from build123d import *

# Parameters (mm, degrees)
SKETCH1_R           = 28
BOSS_EXTRUDE1_DEPTH = 15
HOLE1_D             = 17
HOLE2_D             = 5.5
HOLE2_CBORE_D       = 10
HOLE2_CBORE_DEPTH   = 7
CHAMFER1_SIZE       = 1


with BuildPart() as part:
    # Sketch1 → Boss-Extrude1 (new body)
    with BuildSketch(Plane.XY):
        Circle(SKETCH1_R)
    extrude(amount=BOSS_EXTRUDE1_DEPTH)

    # Hole1 (through all)
    with Locations(Plane.XY.offset(15)):
        with Locations((0, 0)):
            Hole(HOLE1_D / 2)

    # Hole2 (through all)
    with Locations(Plane.XY.offset(15)):
        with Locations((-20, 0), (20, 0)):
            CounterBoreHole(HOLE2_D / 2, HOLE2_CBORE_D / 2, HOLE2_CBORE_DEPTH)

    # Chamfer1
    chamfer1_edges = [part.edges().sort_by_distance(p)[0] for p in [
        (-28, 0, 0),
        (-28, 0, 15),
        (8.5, 0, 15),
        (8.5, 0, 0),
    ]]
    chamfer(chamfer1_edges, length=CHAMFER1_SIZE)


solid = part.part
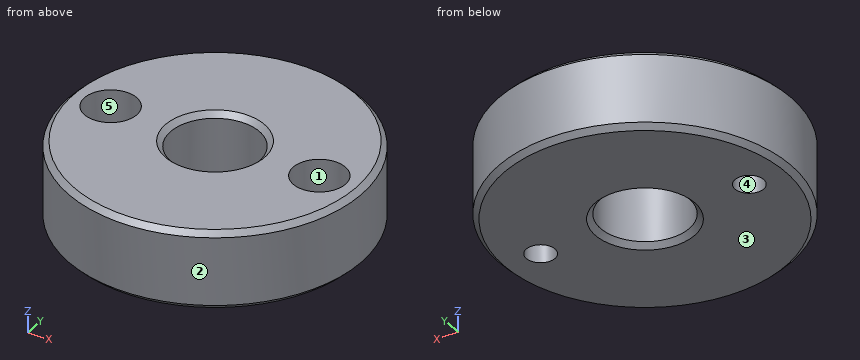
For this review, take the finished solid that the model builds, in its own axes (mm). Face numbers are marked on the shaded views. A direction names the side the tool comes from. Give positions to 0.01 mm unless a question says otherwise; leave off trailing zeros. Loops run counter-clockwise (first coordinate to the right, second up) from the corner with the lowest first, then second, coordinate; pieces in that order, holes last.
Item 1: For line 1 along Y through (x, z) = (0, 8.5); line 2 along X through (y, z) = (7.5, 9.5); line 3 along Y through (x, z) = (-20, 12), list the stretches that pass through material, from the lowest coordinate up.
Item 2: Draft analysis for pull direction X (two halves, no side actions). For the marked faces 1, 2 and 3, state which applies: +X half, -X half, draft (parallel to the pull), parting line (faces both ways), or undercut.
Item 3: Take a section at B-B, the plane x = 0. State the section outline as (y, z) points, and give its area (3 significant figures).
Item 4: Take a section at C-C, the plane z = 11. State the section outline as (x, y) points, and give its area (3 significant figures).
Item 5: Tool access review of the marked faces 4 and 5: name each direction out of +Z, -Z, +X, -X, +Y, -Y from which nothing blocks a thin tool from reaching the whole face with its end or side.
Item 6: Take a section at A-A, the plane y = 0. Give the number of separate pieces and of enclosed holes in the cut face, and give its area (3 significant figures).
Item 7: Insertion check: pin 1 (6.5 mm diameter, centred on x = -20, y = 0, fed in from +Z); pin 2 (3 mm diameter, centred on y = -12, z = 10.5, fed in from -X); pin 3 (2 mm diameter, centred on y = 2.5, z = 1.5, fed in from -X). Each pin has a flat end and moves straight along its axis. Give the tip position at first contact, or say it passes through.
Calculated:
1. line 1: y = -28 to -8.5, 8.5 to 28
1. line 2: x = -26.98 to -4, 4 to 26.98
1. line 3: y = -19.6 to -5, 5 to 19.6
2. face 1: undercut
2. face 2: parting line
2. face 3: draft
3. outline: (-28, 1) - (-27, 0) - (-9.5, 0) - (-8.5, 1) - (-8.5, 14) - (-9.5, 15) - (-27, 15) - (-28, 14) - close; (8.5, 1) - (9.5, 0) - (27, 0) - (28, 1) - (28, 14) - (27, 15) - (9.5, 15) - (8.5, 14) - close
3. area: 581 mm2
4. outline: circle Ø56 at (0, 0); hole circle Ø10 at (-20, 0); hole circle Ø17 at (0, 0); hole circle Ø10 at (20, 0)
4. area: 2,080 mm2
5. face 4: +Z, -Z
5. face 5: +Z
6. separate pieces: 4
6. enclosed holes: 0
6. area: 353 mm2
7. pin 1: stops at z = 8
7. pin 2: stops at x = -25.96
7. pin 3: stops at x = -27.96
